```python
from build123d import *

# Parameters (mm, degrees)
SKETCH1_W                                    = 120
SKETCH1_H                                    = 60
BOSS_EXTRUDE1_DEPTH                          = 10
SKETCH2_R                                    = 14.5
CUT_EXTRUDE1_DEPTH                           = 10
CBORE_FOR_M8_SLOTTED_CHEESE_HEAD_SCR_2_COUNT = 2
CBORE_FOR_M8_SLOTTED_CHEESE_HEAD_SCR_2_PITCH = 56.568542495
CBORE_FOR_M8_SLOTTED_CHEESE_HEAD_SCR_3_COUNT = 2
CBORE_FOR_M8_SLOTTED_CHEESE_HEAD_SCR_3_PITCH = 40
CBORE_FOR_M8_SLOTTED_CHEESE_HEAD_SCR_4_COUNT = 2
CBORE_FOR_M8_SLOTTED_CHEESE_HEAD_SCR_4_PITCH = 40
CBORE_FOR_M5_SLOTTED_CHEESE_HEAD_SCR_2_COUNT = 2
CBORE_FOR_M5_SLOTTED_CHEESE_HEAD_SCR_2_PITCH = 45
CBORE_FOR_M5_SLOTTED_CHEESE_HEAD_SCR_3_COUNT = 2
CBORE_FOR_M5_SLOTTED_CHEESE_HEAD_SCR_3_PITCH = 107
CBORE_FOR_M5_SLOTTED_CHEESE_HEAD_SCR_4_COUNT = 2
CBORE_FOR_M5_SLOTTED_CHEESE_HEAD_SCR_4_PITCH = 116.077560278
M3_TAPPED_HOLE1_D                            = 2.5
M3_TAPPED_HOLE1_DEPTH                        = 12
M3_TAPPED_HOLE1_TIP                          = 0.751075774
CHAMFER1_SIZE                                = 0.5


with BuildPart() as part:
    # Sketch1 → Boss-Extrude1 (new body)
    with BuildSketch(Plane(origin=(0, 0, 0), x_dir=(1, 0, 0), z_dir=(0, 1, 0))):
        with Locations((60, 30)):
            Rectangle(SKETCH1_W, SKETCH1_H)
    extrude(amount=BOSS_EXTRUDE1_DEPTH)

    # Sketch2 → Cut-Extrude1 (cut)
    with BuildSketch(Plane(origin=(0, 10, 0), x_dir=(1, 0, 0), z_dir=(0, 1, 0))):
        with Locations(Location((60, 30, 0), (0, 0, 270))):
            Circle(SKETCH2_R)
    extrude(amount=-CUT_EXTRUDE1_DEPTH, mode=Mode.SUBTRACT)

    # Sketch5 → CBORE for M8 Slotted cheese head screws1 (revolve, cut)
    with BuildSketch(Plane(origin=(80, 10, -10), x_dir=(0, 0, 1), z_dir=(1, 0, 0))):
        Polygon((0, 0), (0, 10), (4.5, 10), (4.5, 6), (7.5, 6), (7.5, 0.025), (7.525, 0), align=None)
    cbore_for_m8_slotted_cheese_head_screws1 = revolve(axis=Axis((80, 16.35, -10), (0, -1, 0)), mode=Mode.SUBTRACT)

    # CBORE for M8 Slotted cheese head scr 2: CBORE for M8 Slotted cheese head screws1 ×2
    with Locations(*[Vector(-0.7071067811865476, 0, -0.7071067811865476) * (i * CBORE_FOR_M8_SLOTTED_CHEESE_HEAD_SCR_2_PITCH) for i in range(1, CBORE_FOR_M8_SLOTTED_CHEESE_HEAD_SCR_2_COUNT)]):
        add(cbore_for_m8_slotted_cheese_head_screws1, mode=Mode.SUBTRACT)

    # CBORE for M8 Slotted cheese head scr 3: CBORE for M8 Slotted cheese head screws1 ×2
    with Locations(*[(0, 0, -i * CBORE_FOR_M8_SLOTTED_CHEESE_HEAD_SCR_3_PITCH) for i in range(1, CBORE_FOR_M8_SLOTTED_CHEESE_HEAD_SCR_3_COUNT)]):
        add(cbore_for_m8_slotted_cheese_head_screws1, mode=Mode.SUBTRACT)

    # CBORE for M8 Slotted cheese head scr 4: CBORE for M8 Slotted cheese head screws1 ×2
    with Locations(*[(-i * CBORE_FOR_M8_SLOTTED_CHEESE_HEAD_SCR_4_PITCH, 0, 0) for i in range(1, CBORE_FOR_M8_SLOTTED_CHEESE_HEAD_SCR_4_COUNT)]):
        add(cbore_for_m8_slotted_cheese_head_screws1, mode=Mode.SUBTRACT)

    # Sketch7 → CBORE for M5 Slotted cheese head screws1 (revolve, cut)
    with BuildSketch(Plane(origin=(6.5, 0, -7.5), x_dir=(0, 0, -1), z_dir=(1, 0, 0))):
        Polygon((0, 0), (0, 10), (2.75, 10), (2.75, 5.7), (5, 5.7), (5, 0.025), (5.025, 0), align=None)
    cbore_for_m5_slotted_cheese_head_screws1 = revolve(axis=Axis((6.5, -6.35, -7.5), (0, 1, 0)), mode=Mode.SUBTRACT)

    # CBORE for M5 Slotted cheese head scr 2: CBORE for M5 Slotted cheese head screws1 ×2
    with Locations(*[(0, 0, -i * CBORE_FOR_M5_SLOTTED_CHEESE_HEAD_SCR_2_PITCH) for i in range(1, CBORE_FOR_M5_SLOTTED_CHEESE_HEAD_SCR_2_COUNT)]):
        add(cbore_for_m5_slotted_cheese_head_screws1, mode=Mode.SUBTRACT)

    # CBORE for M5 Slotted cheese head scr 3: CBORE for M5 Slotted cheese head screws1 ×2
    with Locations(*[(i * CBORE_FOR_M5_SLOTTED_CHEESE_HEAD_SCR_3_PITCH, 0, 0) for i in range(1, CBORE_FOR_M5_SLOTTED_CHEESE_HEAD_SCR_3_COUNT)]):
        add(cbore_for_m5_slotted_cheese_head_screws1, mode=Mode.SUBTRACT)

    # CBORE for M5 Slotted cheese head scr 4: CBORE for M5 Slotted cheese head screws1 ×2
    with Locations(*[Vector(0.9217974580453662, 0, -0.3876718281499204) * (i * CBORE_FOR_M5_SLOTTED_CHEESE_HEAD_SCR_4_PITCH) for i in range(1, CBORE_FOR_M5_SLOTTED_CHEESE_HEAD_SCR_4_COUNT)]):
        add(cbore_for_m5_slotted_cheese_head_screws1, mode=Mode.SUBTRACT)

    # M3 Tapped Hole1
    with Locations(Plane.XY):
        with Locations((20, 5), (100, 5)):
            Hole(M3_TAPPED_HOLE1_D / 2, depth=M3_TAPPED_HOLE1_DEPTH)
            with Locations((0, 0, -(M3_TAPPED_HOLE1_DEPTH + M3_TAPPED_HOLE1_TIP / 2))):  # 118° drill point
                Cone(0, M3_TAPPED_HOLE1_D / 2, M3_TAPPED_HOLE1_TIP, mode=Mode.SUBTRACT)

    # Chamfer1
    chamfer1_edges = [part.edges().sort_by_distance(p)[0] for p in [
        (120, 10, -30),
        (60, 10, -60),
        (0, 10, -30),
        (60, 0, -60),
        (120, 0, -30),
        (60, 0, 0),
        (0, 0, -30),
        (0, 5, -60),
        (120, 5, -60),
        (120, 5, 0),
        (0, 5, 0),
        (60, 10, 0),
    ]]
    chamfer(chamfer1_edges, length=CHAMFER1_SIZE)


solid = part.part
```
For this review, take the finished solid that the model builds, in its own axes (mm). A direction names the side the tool comes from. Round coordinates to 2 decimals unless told otherwise and drop trailing zeros. Loops run counter-clockwise (first coordinate to the right, second up) from the corner with the lowest first, then second, coordinate; pieces in that order, holes last.
Q1. Machinability: for faces 1 (the face through (0, 5, -30)), 2 (the face through (116, 5.7, -50)), 3 (the face through (98.845, 4.521, -6.084)), 4 (the face through (32.564, 7.029, -10.976)), which of the approach directions +Z, -Z, +X, -X, +Y, -Y give a long, thin tool a straight path to every point of the face, cutting with its end or side? Answer none if there is none.
Result sheet:
face 1: +Z, -Z, -X, +Y, -Y
face 2: -Y
face 3: +Z
face 4: +Y
Q2. Add section C-C on x = 113.5. Write out the cut boundary in (y, z) (3 decimals), plus the area to 3 significant figures.
Result sheet:
outline: (0, -59.5) - (0.5, -60) - (9.5, -60) - (10, -59.5) - (10, -55.25) - (5.7, -55.25) - (5.7, -57.5) - (0.025, -57.5) - (0, -57.525) - close; (0, -47.475) - (0.025, -47.5) - (5.7, -47.5) - (5.7, -49.75) - (10, -49.75) - (10, -10.25) - (5.7, -10.25) - (5.7, -12.5) - (0.025, -12.5) - (0, -12.525) - close; (0, -2.475) - (0.025, -2.5) - (5.7, -2.5) - (5.7, -4.75) - (10, -4.75) - (10, -0.5) - (9.5, 0) - (0.5, 0) - (0, -0.5) - close
area: 438 mm2
Q3. Add section A-A on z = -20. Write out the cut boundary in (x, y), plus the area to 4 significant figures.
Result sheet:
outline: (0, 0.5) - (0.5, 0) - (49.5, 0) - (49.5, 10) - (0.5, 10) - (0, 9.5) - close; (70.5, 0) - (119.5, 0) - (120, 0.5) - (120, 9.5) - (119.5, 10) - (70.5, 10) - close
area: 989.5 mm2
Q4. Insertion check: pin 1 Ø4.5 at (x, z) = (113.5, -7.5) entering from +Y; pin 2 Ø14.5 at (x, z) = (40, -50) entering from +Y; pin 3 Ø2 at (x, y) = (100, 5) entering from +Z; pin 4 Ø6 at (x, z) = (6.5, -52.5) entering from -Y. Each pin has a flat end and moves straight along its axis. Give the tip position at first contact, or say it passes through.
Result sheet:
pin 1: passes through
pin 2: stops at y = 4
pin 3: stops at z = -12.15
pin 4: stops at y = 5.7
Q5. To check wall thickness, follow line 1 along Z through (x, y) = (6.5, 7.7); line 2 along X through (y, z) = (6.75, -56); line 3 along Z through (x, y) = (6.5, 1.85). State the ranges of each line that lie inside material, in increasing order.
Result sheet:
line 1: z = -60 to -55.25, -49.75 to -10.25, -4.75 to 0
line 2: x = 0 to 35.5, 44.5 to 75.5, 84.5 to 120
line 3: z = -60 to -57.5, -47.5 to -12.5, -2.5 to 0
Q6. Add section B-B on y = 2. Give the number of separate pieces and of enclosed holes in the cut face, plus the area to 3 significant figures.
Result sheet:
separate pieces: 1
enclosed holes: 9
area: 5,970 mm2
Q7. Add section D-D on x = 51.5. Write out the cut boundary in (y, z).
Result sheet:
outline: (0, -59.5) - (0.5, -60) - (9.5, -60) - (10, -59.5) - (10, -41.75) - (0, -41.75) - close; (0, -18.25) - (10, -18.25) - (10, -0.5) - (9.5, 0) - (0.5, 0) - (0, -0.5) - close
Q8. Mouldability with a two-part tool opening along Z and no side actions: class faces 5 (the face through (36.206, 2.028, -47.581)), 6 (the face through (20.21, 5.07, -12.62)), 7 (the face through (46, 0, -37)), 8 (the face through (5, 2.82, -12.27)) as +Z half, -Z half, draft (parallel to the pull), parting line (faces both ways), or undercut.
Result sheet:
face 5: undercut
face 6: +Z half
face 7: draft
face 8: undercut
